For this review, take the finished solid that the model builds, in its own axes (mm). A direction names the side the tool comes from. Coordinates: 2 decimals unless noted, no trailing zeros. Loops run counter-clockwise (first coordinate to the right, second up) from the corner with the lowest first, then second, coordinate; pieces in that order, holes last. Notation, with made-up numbers: (85.5, 63) -> (138.5, 63) arc R20 ccw to (138.5, 91) -> close; hole circle Ø7 at (36, 66). An arc over 180 degrees is marked (long way). Answer in a Markdown table with one row per item.
from build123d import *

# Parameters (mm, degrees)
SKETCH_1_W             = 112
SKETCH_1_H             = 68
EXTRUDE_1_DEPTH        = 12
SKETCH_2_W             = 40
SKETCH_2_H             = 30
CUT_EXTRUDE_1_DEPTH    = 12
HOLE_WIZARD_M12_1_D    = 10.2
CHAMFER_1_SIZE         = 3
FILLET_1_R             = 3
HOLE_WIZARD_M6_1_D     = 5
HOLE_WIZARD_M6_1_DEPTH = 15
HOLE_WIZARD_M6_1_TIP   = 1.502151548
HOLE_WIZARD_M5_1_D     = 4.2
HOLE_WIZARD_M5_1_DEPTH = 12.4
HOLE_WIZARD_M5_1_TIP   = 1.2618073


with BuildPart() as part:
    # 草图1 → 凸台-拉伸1 (new body)
    with BuildSketch(Plane.XY):
        with Locations((56, 34)):
            Rectangle(SKETCH_1_W, SKETCH_1_H)
    extrude(amount=EXTRUDE_1_DEPTH)

    # 草图2 → 切除-拉伸1 (cut)
    with BuildSketch(Plane.XY.offset(12)):
        with Locations((20, 15)):
            Rectangle(SKETCH_2_W, SKETCH_2_H)
    cut_extrude_1 = extrude(amount=-CUT_EXTRUDE_1_DEPTH, mode=Mode.SUBTRACT)

    # 镜向1: 切除-拉伸1 across plane
    add(cut_extrude_1.mirror(Plane.ZY.offset(-56)), mode=Mode.SUBTRACT)

    # M12 螺纹孔1 (through all)
    with Locations(Plane.XY.offset(12)):
        with Locations((56, 17)):
            Hole(HOLE_WIZARD_M12_1_D / 2)

    # 倒角1
    chamfer_1_edges = [part.edges().sort_by_distance(p)[0] for p in [
        (0, 30, 6),
        (40, 0, 6),
        (112, 30, 6),
        (72, 0, 6),
    ]]
    chamfer(chamfer_1_edges, length=CHAMFER_1_SIZE)

    # 圆角1
    fillet_1_edges = [part.edges().sort_by_distance(p)[0] for p in [
        (40, 30, 6),
        (72, 30, 6),
    ]]
    fillet(fillet_1_edges, radius=FILLET_1_R)

    # M6 螺纹孔1
    with Locations(Plane(origin=(0, 68, 0), x_dir=(1, 0, 0), z_dir=(0, 1, 0))):
        with Locations((101, -6), (56, -6), (11, -6)):
            Hole(HOLE_WIZARD_M6_1_D / 2, depth=HOLE_WIZARD_M6_1_DEPTH)
            with Locations((0, 0, -(HOLE_WIZARD_M6_1_DEPTH + HOLE_WIZARD_M6_1_TIP / 2))):  # 118° drill point
                Cone(0, HOLE_WIZARD_M6_1_D / 2, HOLE_WIZARD_M6_1_TIP, mode=Mode.SUBTRACT)

    # M5 螺纹孔1
    with Locations(Plane(origin=(0, 0, 0), x_dir=(-1, 0, 0), z_dir=(0, -1, 0))):
        with Locations((-63.5, -6), (-48.5, -6)):
            Hole(HOLE_WIZARD_M5_1_D / 2, depth=HOLE_WIZARD_M5_1_DEPTH)
            with Locations((0, 0, -(HOLE_WIZARD_M5_1_DEPTH + HOLE_WIZARD_M5_1_TIP / 2))):  # 118° drill point
                Cone(0, HOLE_WIZARD_M5_1_D / 2, HOLE_WIZARD_M5_1_TIP, mode=Mode.SUBTRACT)


solid = part.part
Item 1: Insertion check: pin 1 (6 mm diameter, centred on x = 11, z = 6, fed in from +Y); pin 2 (8 mm diameter, centred on x = 56, y = 17, fed in from -Z); pin 3 (3.5 mm diameter, centred on x = 96.5, z = 5, fed in from -Y); pin 4 (4 mm diameter, centred on y = 24.5, z = 6.5, fed in from -X). Each pin has a flat end and moves straight along its axis. Give the tip position at first contact, or say it passes through.
Worked answers:
| item | result |
|---|---|
| pin 1 | y = 68 |
| pin 2 | through |
| pin 3 | y = 30 |
| pin 4 | x = 40 |
Item 2: Take a section at A-A, the plane y = 55.5. State the section outline as (x, z) points.
Worked answers:
| item | result |
|---|---|
| outline | (0, 0) -> (112, 0) -> (112, 12) -> (0, 12) -> close; hole circle Ø5 at (11, 6); hole circle Ø5 at (56, 6); hole circle Ø5 at (101, 6) |
Item 3: Take a section at C-C, the plane x = 84. State the section outline as (y, z) points.
Worked answers:
| item | result |
|---|---|
| outline | (30, 0) -> (68, 0) -> (68, 12) -> (30, 12) -> close |
Item 4: For faces 4 (the cylindrical face through (39.1, 29.14, 5.92)), 5 (the cylindrical face through (13.5, 60.4, 5.9)), 6 (the flat face through (72, 15, 6)), list the 3-axis set-ups (+Z, -Z, +X, -X, +Y, -Y) from which the entire face can be reached by the end or side of a thin tool; tool diameter is ignored.
Worked answers:
| item | result |
|---|---|
| face 4 | +Z, -Z, -X, -Y |
| face 5 | +Y |
| face 6 | +Z, -Z, +X, -Y |
Item 5: Take a section at B-B, the plane y = 5. State the section outline as (x, z) points, and give its area (3 significant figures).
Worked answers:
| item | result |
|---|---|
| outline | (40, 0) -> (72, 0) -> (72, 12) -> (40, 12) -> close; hole circle Ø4.2 at (48.5, 6); hole circle Ø4.2 at (63.5, 6) |
| area | 356 mm² |
Item 6: The part is to be moulded in two halves that separate along X. For faces 1 (the conical face through (10.68, 51.759, 5.707)), 2 (the flat face through (56, 0, 6)), 3 (the flat face through (110, 31, 6)), say which applies: +X half, -X half, draft (parallel to the pull), parting line (faces both ways), or undercut.
Worked answers:
| item | result |
|---|---|
| face 1 | undercut |
| face 2 | draft |
| face 3 | +X half |
Item 7: For L1, parallel to Z at x = 11, y = 59.75; L2, parallel to Y at x = 78, z = 8.5; L3, parallel to X at y = 62, z = 7, list the stretches that pass through material, from the lowest coordinate up.
Worked answers:
| item | result |
|---|---|
| L1 | 0 to 3.5, 8.5 to 12 |
| L2 | 30 to 68 |
| L3 | 0 to 8.71, 13.29 to 53.71, 58.29 to 98.71, 103.29 to 112 |
